The model under review builds one solid part; all positions refer to its coordinate system, in mm. Coordinates: 2 decimals unless noted, no trailing zeros. Order: outer loops, then holes, each group sorted by start corner. A loop starts at its lowest first (then second) coordinate and runs counter-clockwise, first axis right, second up. Notation, with made-up numbers: M 73.5,-2 L 111.5,-2 A24 cw 111.5,15 Z; hole C 24,5.25 d8. An arc over 180 degrees is marked long. Answer in a Markdown table with one row per item.
from build123d import *

# Parameters (mm, degrees)
SKETCH1_R           = 2.25
SKETCH1_R_2         = 1
BOSS_EXTRUDE1_DEPTH = 2.5
CHAMFER1_SIZE       = 0.2
SKETCH2_W           = 0.8
SKETCH2_H           = 2.25


with BuildPart() as part:
    # Sketch1 → Boss-Extrude1 (new, symmetric)
    with BuildSketch(Plane.XY):
        Circle(SKETCH1_R)
        Circle(SKETCH1_R_2, mode=Mode.SUBTRACT)
    extrude(amount=BOSS_EXTRUDE1_DEPTH, both=True)

    # Chamfer1
    chamfer1_edges = [part.edges().sort_by_distance(p)[0] for p in [
        (-2.25, 0, -2.5),
        (-2.25, 0, 2.5),
        (-1, 0, -2.5),
        (-1, 0, 2.5),
    ]]
    chamfer(chamfer1_edges, length=CHAMFER1_SIZE)

    # Sketch2 → M2 Tapped Hole1 (revolve, cut)
    with BuildSketch(Plane(origin=(0, 0, 1), x_dir=(0, 0, -1), z_dir=(1, 0, 0))):
        with Locations((0.4, 1.125)):
            Rectangle(SKETCH2_W, SKETCH2_H)
    revolve(axis=Axis((0, -6.35, 1), (0, 1, 0)), mode=Mode.SUBTRACT)


solid = part.part
(1) Take a section at B-B (x = 0). Write out the cut boundary in (y, z), then the cut area to 3 significant figures.
Report:
| item | result |
|---|---|
| outline | M -2.25,-2.3 L -2.05,-2.5 L -1.2,-2.5 L -1,-2.3 L -1,2.3 L -1.2,2.5 L -2.05,2.5 L -2.25,2.3 Z; M 1,-2.3 L 1.2,-2.5 L 2.05,-2.5 L 2.25,-2.3 L 2.25,0.2 L 1,0.2 Z; M 1,1.8 L 2.25,1.8 L 2.25,2.3 L 2.05,2.5 L 1.2,2.5 L 1,2.3 Z |
| area | 10.3 mm^2 |
(2) Take a section at C-C (z = 1.55). Write out the cut boundary in (x, y), then the cut area to 3 significant figures.
Report:
| item | result |
|---|---|
| outline | M -0.58,0.81 L -0.58,2.17 A2.25 ccw long 0.58,2.17 L 0.58,0.81 A1 cw long Z |
| area | 11.3 mm^2 |
(3) Take a section at A-A (y = 0). Write out the cut boundary in (x, z), then the cut area to 3 significant figures.
Report:
| item | result |
|---|---|
| outline | M -2.25,-2.3 L -2.05,-2.5 L -1.2,-2.5 L -1,-2.3 L -1,2.3 L -1.2,2.5 L -2.05,2.5 L -2.25,2.3 Z; M 1,-2.3 L 1.2,-2.5 L 2.05,-2.5 L 2.25,-2.3 L 2.25,2.3 L 2.05,2.5 L 1.2,2.5 L 1,2.3 Z |
| area | 12.3 mm^2 |
(4) To check wall thickness, follow line 1 (Y direction, x = 0, z = -0.05); line 2 (Y direction, x = -0.8, z = -2.05); line 3 (X direction, y = 1.35, z = 1). State the ranges of each line that lie inside material, in increasing order. Write a range as [from, to].
Report:
| item | result |
|---|---|
| line 1 | [-2.25, -1], [1, 2.25] |
| line 2 | [-2.1, -0.6], [0.6, 2.1] |
| line 3 | [-1.8, -0.8], [0.8, 1.8] |
(5) The part is to be moulded in two halves that separate along Z. For faces 1 (the cylindrical face through (0, 1.4, 1.8)), 2 (the flat face through (1, -1, 2.5)), 3 (the flat face through (1, -1, -2.5)), say which applies: +Z half, -Z half, draft (parallel to the pull), parting line (faces both ways), or undercut.
Report:
| item | result |
|---|---|
| face 1 | undercut |
| face 2 | +Z half |
| face 3 | -Z half |
(6) Take a section at D-D (x = 0.55). State how many separate pieces and enclosed holes the cut face has, then the cut area to 3 significant figures.
Report:
| item | result |
|---|---|
| separate pieces | 3 |
| enclosed holes | 0 |
| area | 11.7 mm^2 |
(7) Insertion check: P1, Ø1, axis at y = 1, z = 0.5, coming from the -X side. The pin has a flat end and moves straight along its axis. Give the tip position at first contact, or say it passes through.
Report:
| item | result |
|---|---|
| P1 | x = -2.19 |
